Here's how the part is built. I have some questions about the finished solid (model axes, mm). Face numbers are marked on the shaded views. Round coordinates to 2 decimals unless told otherwise and drop trailing zeros. Loops run counter-clockwise (first coordinate to the right, second up) from the corner with the lowest first, then second, coordinate; pieces in that order, holes last. Notation, with made-up numbers: (9.25, 85) - (36.25, 85) arc R23 cw to (36.25, 115) - close; hole circle Ø5 at (44.25, 10). An arc over 180 degrees is marked (long way). Answer as a JSON object with one key per item and string values. Group by question number.
1) If I drill on line 1 along Z through (x, y) = (0, -15.5); line 2 along Z through (x, y) = (-9, -18.5), over which ranges is the centre line in solid material (lowest first)? Write a range as [from, to].
2) I want a section at C-C, the plane y = -17.5. Please give me the cut outline in (x, z).
3) I want a section at D-D, the plane x = 11.5. Please give me the cut outline in (y, z).
4) If we mould it in two halves opening along X, with no side actions, what happens to the marked faces 1, 2 and 3? For each: pulls with the +X half, pulls with the -X half, needs draft (parallel to the pull), parting line crosses it, or undercut.
5) I want a section at B-B, the plane x = -4. Please give me the cut outline in (y, z), then the cut area to 3 significant figures.
6) I want a section at A-A, the plane y = 16. Please give me the cut outline in (x, z), then the cut area to 3 significant figures.
7) Will these pins go through, and if not, where does the flat tip stop? P1, Ø1, axis at x = 1.5, y = 9.5, coming from the -Z side; P2, Ø8, axis at x = 1, y = -16.5, coming from the +Z side; P3, Ø1.6, axis at x = 17.5, z = -5.5, coming from the +Y side.
from build123d import *

# Parameters (mm, degrees)
SKETCH_1_W          = 36
SKETCH_1_H          = 43
EXTRUDE_1_DEPTH     = 6
SKETCH_2_W          = 12
SKETCH_2_H          = 43
CUT_EXTRUDE_1_DEPTH = 1.5
SKETCH_3_W          = 30.5
SKETCH_3_H          = 43
CUT_EXTRUDE_2_DEPTH = 1.5
SKETCH_4_W          = 36
SKETCH_4_H          = 35
CUT_EXTRUDE_3_DEPTH = 1.5


with BuildPart() as part:
    # 草图1 → 凸台-拉伸1 (new, symmetric)
    with BuildSketch(Plane.XY):
        Rectangle(SKETCH_1_W, SKETCH_1_H)
    extrude(amount=EXTRUDE_1_DEPTH, both=True)

    # 草图2 → 切除-拉伸1 (cut)
    with BuildSketch(Plane.XY.offset(6)):
        Rectangle(SKETCH_2_W, SKETCH_2_H)
    extrude(amount=-CUT_EXTRUDE_1_DEPTH, mode=Mode.SUBTRACT)

    # 草图3 → 切除-拉伸2 (cut)
    with BuildSketch(Plane(origin=(0, 0, -6), x_dir=(-1, 0, 0), z_dir=(0, 0, -1))):
        Rectangle(SKETCH_3_W, SKETCH_3_H)
    extrude(amount=-CUT_EXTRUDE_2_DEPTH, mode=Mode.SUBTRACT)

    # 草图4 → 切除-拉伸3 (cut)
    with BuildSketch(Plane(origin=(0, 0, -6), x_dir=(-1, 0, 0), z_dir=(0, 0, -1))):
        with Locations((0, 4)):
            Rectangle(SKETCH_4_W, SKETCH_4_H)
    extrude(amount=-CUT_EXTRUDE_3_DEPTH, mode=Mode.SUBTRACT)


solid = part.part
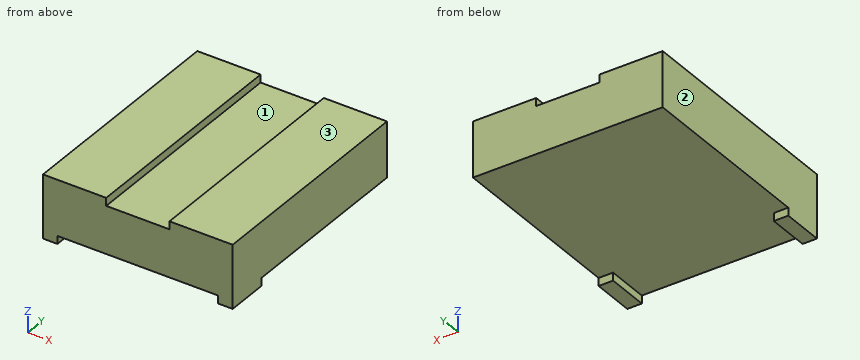
Outcome:
{
 "1": {"line 1": "[-4.5, 4.5]", "line 2": "[-4.5, 6]"},
 "2": {"outline": "(-18, -6) - (-15.25, -6) - (-15.25, -4.5) - (15.25, -4.5) - (15.25, -6) - (18, -6) - (18, 6) - (6, 6) - (6, 4.5) - (-6, 4.5) - (-6, 6) - (-18, 6) - close"},
 "3": {"outline": "(-21.5, -4.5) - (21.5, -4.5) - (21.5, 6) - (-21.5, 6) - close"},
 "4": {"face 1": "undercut", "face 2": "pulls with the -X half", "face 3": "needs draft"},
 "5": {"outline": "(-21.5, -4.5) - (21.5, -4.5) - (21.5, 4.5) - (-21.5, 4.5) - close", "area": "387 mm^2"},
 "6": {"outline": "(-18, -4.5) - (18, -4.5) - (18, 6) - (6, 6) - (6, 4.5) - (-6, 4.5) - (-6, 6) - (-18, 6) - close", "area": "360 mm^2"},
 "7": {"P1": "z = -4.5", "P2": "z = 4.5", "P3": "y = -13.5"}
}
